Input: dimensioned drawing with shaded views. Units: mm. Origin: part minimum x, y, z. Round coordinates to 2 decimals unless told otherwise and drop trailing zeros. Loops run counter-clockwise (first coordinate to the right, second up) from the corner with the lowest first, then second, coordinate; pieces in that order, holes last. Notation, with made-up numbers: M -12,52.5 L 17,52.5 A17 ccw 17,84.5 Z; hole C 62.25,23 d7. An arc over 180 degrees is marked long. Put each result on its own line as item: value. Start each with the question number.
1) Section B-B on y = 50. Output: boundary loops of the cut face in (x, z), plus the area to 3 significant figures.
2) Line query: probe 1 along X at (y, z) = (50.5, 16.75); probe 2 along Y at (x, z) = (15, 9.5). Output: solid intervals per line, ascending.
3) Pin query (flat end, axial travel): pin 1 (1 mm diameter, centred on y = 18, z = 5, fed in from -X). Return the tip coordinate at first contact, or that it passes through.
4) Section A-A on x = 15. Output: boundary loops of the cut face in (y, z).
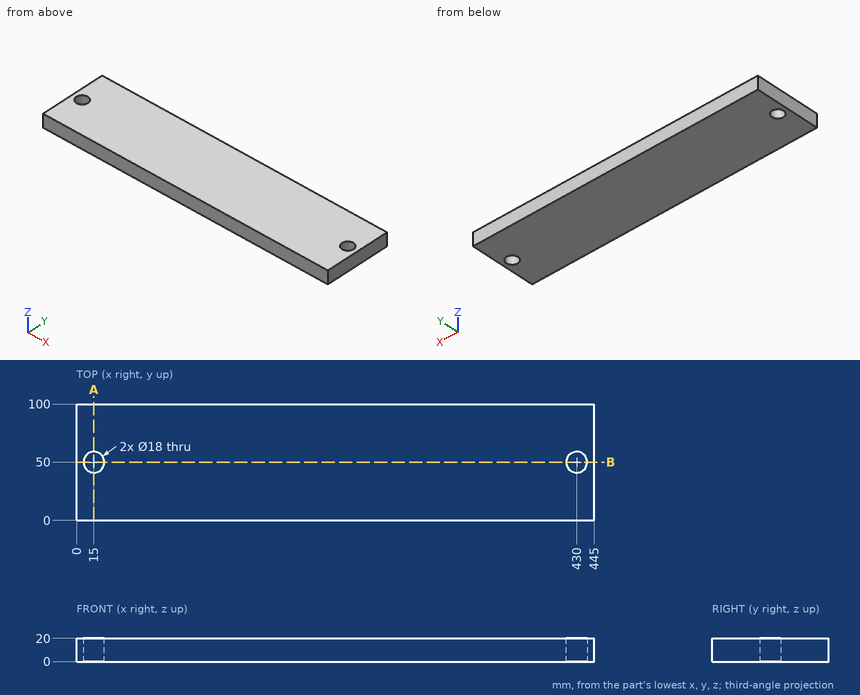
Geometry results:
1. outline: M 0,0 L 6,0 L 6,20 L 0,20 Z; M 24,0 L 421,0 L 421,20 L 24,20 Z; M 439,0 L 445,0 L 445,20 L 439,20 Z
1. area: 8,180 mm²
2. probe 1: x = 0 to 6.01, 23.99 to 421.01, 438.99 to 445
2. probe 2: y = 0 to 41, 59 to 100
3. pin 1: stops at x = 0
4. outline: M 0,0 L 41,0 L 41,20 L 0,20 Z; M 59,0 L 100,0 L 100,20 L 59,20 Z
